from build123d import *

# Parameters (mm, degrees)
SKETCH_1_R      = 15
EXTRUDE_1_DEPTH = 170.5
SKETCH_2_R      = 10
EXTRUDE_2_DEPTH = 10


with BuildPart() as part:
    # 草图1 → 凸台-拉伸1 (new, symmetric)
    with BuildSketch(Plane.XY):
        with Locations(Location((0, 0, 0), (0, 0, 180))):
            Circle(SKETCH_1_R)
    extrude(amount=EXTRUDE_1_DEPTH, both=True)

    # 草图2 → 凸台-拉伸2 (add)
    with BuildSketch(Plane.XY.offset(170.5)):
        Circle(SKETCH_2_R)
    extrude_2 = extrude(amount=EXTRUDE_2_DEPTH)

    # 镜向1: 凸台-拉伸2 across plane
    add(extrude_2.mirror(Plane.XY))


solid = part.part
Read the model definition and answer for the solid it produces. Units are mm, in the model's axes. A direction names the side the tool comes from. Round coordinates to 2 decimals unless told otherwise and drop trailing zeros. Order: outer loops, then holes, each group sorted by start corner. A loop starts at its lowest first (then second) coordinate and runs counter-clockwise, first axis right, second up.
1) Flat-ended cylindrical pins translate along their axes: pin 1 (1.5 mm diameter, centred on x = -4.5, z = -19.5, fed in from +Y); pin 2 (1.5 mm diameter, centred on y = -1, z = 52.5, fed in from +X); pin 3 (3 mm diameter, centred on x = -3.5, z = 64.5, fed in from +Y). Find the tip coordinate at first contact, or state that the pin passes through.
2) The part is cut by section A-A on x = 0. Write down the section's boundary in (y, z), plus the area to 3 significant figures.
3) The part is cut by section C-C on z = -123. Write down the section's boundary in (x, y), plus the area to 3 significant figures.
4) For faces 1 (the face through (-2.17, -9.76, -175.43)), 2 (the face through (-2.17, -9.76, 175.43)), 3 (the face through (0, 0, 180.5)), determine the directions among +Z, -Z, +X, -X, +Y, -Y from which every point of the face is accessible in a straight line to the end or side of a thin tool.
5) Straight lines are drawn through the part: L1, parallel to Z at x = 3, y = 13; L2, parallel to Y at x = 3.75, z = 63; L3, parallel to Y at x = 13.75, z = 118.5. For each, find the intervals that lie inside material, in ascending order.
Resolved:
1. pin 1: stops at y = 14.52
1. pin 2: stops at x = 15
1. pin 3: stops at y = 14.87
2. outline: (-15, -170.5) - (-10, -170.5) - (-10, -180.5) - (10, -180.5) - (10, -170.5) - (15, -170.5) - (15, 170.5) - (10, 170.5) - (10, 180.5) - (-10, 180.5) - (-10, 170.5) - (-15, 170.5) - close
2. area: 10,600 mm2
3. outline: circle Ø30 at (0, 0)
3. area: 707 mm2
4. face 1: -Z
4. face 2: +Z
4. face 3: +Z, +X, -X, +Y, -Y
5. L1: z = -170.5 to 170.5
5. L2: y = -14.52 to 14.52
5. L3: y = -5.99 to 5.99
